```python
from build123d import *

# Parameters (mm, degrees)
SKETCH1_W                                            = 106
SKETCH1_H                                            = 187
BOSS_EXTRUDE1_DEPTH                                  = 9
SKETCH2_R                                            = 30
CUT_EXTRUDE1_DEPTH                                   = 109.973620661
SKETCH3_R                                            = 32.5
CUT_EXTRUDE2_DEPTH                                   = 7
CUT_EXTRUDE3_START                                   = -7
SKETCH4_R                                            = 32.5
CUT_EXTRUDE3_DEPTH                                   = 7
SKETCH5_W                                            = 62
SKETCH5_H                                            = 68
CUT_EXTRUDE4_DEPTH                                   = 109.973620661
FILLET1_R                                            = 2
SKETCH6_W                                            = 9
SKETCH6_H                                            = 87
CUT_EXTRUDE5_DEPTH                                   = 142.630681704
M4_TAPPED_HOLE1_D                                    = 3.3
M4_TAPPED_HOLE2_D                                    = 3.3
M3_TAPPED_HOLE1_D                                    = 2.5
M3_TAPPED_HOLE1_DEPTH                                = 7.5
M3_TAPPED_HOLE1_TIP                                  = 0.751075774
CHAMFER1_SIZE                                        = 5
HOLE_SIZE_PER_SOCKET_HEAD_CAP_SCREW_TYPE_D           = 4.5
HOLE_SIZE_PER_SOCKET_HEAD_CAP_SCREW_TYPE_CBORE_D     = 8
HOLE_SIZE_PER_SOCKET_HEAD_CAP_SCREW_TYPE_CBORE_DEPTH = 5
HOLE_SIZE_PER_SOCKET_HEAD_CAP_SCREW_2_D              = 5.5
HOLE_SIZE_PER_SOCKET_HEAD_CAP_SCREW_2_CBORE_D        = 10
HOLE_SIZE_PER_SOCKET_HEAD_CAP_SCREW_2_CBORE_DEPTH    = 9
M5_TAPPED_HOLE1_D                                    = 4.2
M5_TAPPED_HOLE1_DEPTH                                = 12.4
M5_TAPPED_HOLE1_TIP                                  = 1.2618073
M4_TAPPED_HOLE3_D                                    = 3.3
M4_TAPPED_HOLE3_DEPTH                                = 12.1
M4_TAPPED_HOLE3_TIP                                  = 0.991420021


with BuildPart() as part:
    # Sketch1 → Boss-Extrude1 (new, symmetric)
    with BuildSketch(Plane.XY):
        Rectangle(SKETCH1_W, SKETCH1_H)
    extrude(amount=BOSS_EXTRUDE1_DEPTH, both=True)

    # Sketch2 → Cut-Extrude1 (cut, through all)
    with BuildSketch(Plane(origin=(0, 0, -9), x_dir=(-1, 0, 0), z_dir=(0, 0, -1))):
        with Locations((0, 40.5)):
            Circle(SKETCH2_R)
    extrude(amount=-CUT_EXTRUDE1_DEPTH, mode=Mode.SUBTRACT)

    # Sketch3 → Cut-Extrude2 (cut)
    with BuildSketch(Plane.XY.offset(9)):
        with Locations((0, 40.5)):
            Circle(SKETCH3_R)
    extrude(amount=-CUT_EXTRUDE2_DEPTH, mode=Mode.SUBTRACT)

    # Sketch4 → Cut-Extrude3 (cut)
    with BuildSketch(Plane(origin=(0, 0, -9), x_dir=(-1, 0, 0), z_dir=(0, 0, -1)).offset(CUT_EXTRUDE3_START)):
        with Locations(Location((0, 40.5, 0), (0, 0, 180))):
            Circle(SKETCH4_R)
    extrude(amount=CUT_EXTRUDE3_DEPTH, mode=Mode.SUBTRACT)

    # Sketch5 → Cut-Extrude4 (cut, through all)
    with BuildSketch(Plane.XY.offset(9)):
        with Locations((0, -40.5)):
            Rectangle(SKETCH5_W, SKETCH5_H)
    extrude(amount=-CUT_EXTRUDE4_DEPTH, mode=Mode.SUBTRACT)

    # Fillet1
    fillet1_edges = [part.edges().sort_by_distance(p)[0] for p in [
        (-31, -74.5, 0),
        (-31, -6.5, 0),
        (31, -6.5, 0),
        (31, -74.5, 0),
    ]]
    fillet(fillet1_edges, radius=FILLET1_R)

    # Sketch6 → Cut-Extrude5 (cut, through all)
    with BuildSketch(Plane(origin=(53, 0, 0), x_dir=(0, 0, -1), z_dir=(1, 0, 0))):
        with Locations((-4.5, -50)):
            Rectangle(SKETCH6_W, SKETCH6_H)
    extrude(amount=-CUT_EXTRUDE5_DEPTH, mode=Mode.SUBTRACT)

    # M4 Tapped Hole1 (through all)
    with Locations(Plane.XY):
        with Locations((36, -24), (36, -59), (-36, -59), (-36, -24)):
            Hole(M4_TAPPED_HOLE1_D / 2)

    # M4 Tapped Hole2 (through all)
    with Locations(Plane.XY):
        with Locations((-8, -83.5), (8, -83.5)):
            Hole(M4_TAPPED_HOLE2_D / 2)

    # M3 Tapped Hole1
    with Locations(Plane.XY.offset(9)):
        with Locations((-38, 45.5), (-38, 37.5), (-38, -0.5)):
            Hole(M3_TAPPED_HOLE1_D / 2, depth=M3_TAPPED_HOLE1_DEPTH)
            with Locations((0, 0, -(M3_TAPPED_HOLE1_DEPTH + M3_TAPPED_HOLE1_TIP / 2))):  # 118° drill point
                Cone(0, M3_TAPPED_HOLE1_D / 2, M3_TAPPED_HOLE1_TIP, mode=Mode.SUBTRACT)

    # Chamfer1
    chamfer1_edges = [part.edges().sort_by_distance(p)[0] for p in [
        (-53, 93.5, 0),
        (53, 93.5, 0),
    ]]
    chamfer(chamfer1_edges, length=CHAMFER1_SIZE)

    # Hole size per socket head cap screw type (through all)
    with Locations(Plane(origin=(0, 0, -9), x_dir=(-1, 0, 0), z_dir=(0, 0, -1))):
        with Locations((-38, 33.5)):
            CounterBoreHole(HOLE_SIZE_PER_SOCKET_HEAD_CAP_SCREW_TYPE_D / 2, HOLE_SIZE_PER_SOCKET_HEAD_CAP_SCREW_TYPE_CBORE_D / 2, HOLE_SIZE_PER_SOCKET_HEAD_CAP_SCREW_TYPE_CBORE_DEPTH)

    # Hole size per socket head cap screw  2 (through all)
    with Locations(Plane.XY.offset(9)):
        with Locations((-47, 9.05741234), (-47, -30.94258766), (-47, -70.94258766), (47, -70.94258766), (47, -30.94258766), (47, 9.05741234)):
            CounterBoreHole(HOLE_SIZE_PER_SOCKET_HEAD_CAP_SCREW_2_D / 2, HOLE_SIZE_PER_SOCKET_HEAD_CAP_SCREW_2_CBORE_D / 2, HOLE_SIZE_PER_SOCKET_HEAD_CAP_SCREW_2_CBORE_DEPTH)

    # M5 Tapped Hole1
    with Locations(Plane.XY.offset(9)):
        with Locations((0, -0.5)):
            Hole(M5_TAPPED_HOLE1_D / 2, depth=M5_TAPPED_HOLE1_DEPTH)
            with Locations((0, 0, -(M5_TAPPED_HOLE1_DEPTH + M5_TAPPED_HOLE1_TIP / 2))):  # 118° drill point
                Cone(0, M5_TAPPED_HOLE1_D / 2, M5_TAPPED_HOLE1_TIP, mode=Mode.SUBTRACT)

    # M4 Tapped Hole3
    with Locations(Plane(origin=(0, 93.5, 0), x_dir=(1, 0, 0), z_dir=(0, 1, 0))):
        with Locations((-35, 0), (35, 0)):
            Hole(M4_TAPPED_HOLE3_D / 2, depth=M4_TAPPED_HOLE3_DEPTH)
            with Locations((0, 0, -(M4_TAPPED_HOLE3_DEPTH + M4_TAPPED_HOLE3_TIP / 2))):  # 118° drill point
                Cone(0, M4_TAPPED_HOLE3_D / 2, M4_TAPPED_HOLE3_TIP, mode=Mode.SUBTRACT)


solid = part.part
```
Can you work these out from the model? Positions are in its coordinate system, mm. A direction names the side the tool comes from. Give positions to 0.01 mm unless a question says otherwise; leave off trailing zeros. Loops run counter-clockwise (first coordinate to the right, second up) from the corner with the lowest first, then second, coordinate; pieces in that order, holes last. Notation, with made-up numbers: M -20.75,45.5 L -4.75,45.5 A21 cw -4.75,63.5 Z; hole C -38.5,81 d6. An arc over 180 degrees is marked long. One line per question, with ' | ' between items. Start each with the question number.
Q1. If we section it at D-D (x = 12.5): Please give me the cut outline in (y, z).
Q2. For faces 1 (the flat face through (1, -80, 0)), 2 (the flat face through (9.5, 11.8, 2)), 3 (the cylindrical face through (38.521, 37.466, -6.535)), 4 (the flat face through (31, -41, -4)), which set-ups out of +Z, -Z, +X, -X, +Y, -Y let a thin tool reach every point of the face, with its end or its side?
Q3. If we section it at C-C (y = 40.5): Please give me the cut outline in (x, z), plus the area to 3 significant figures.
Q4. If we section it at B-B (x = -26): Please give me the cut outline in (y, z).
Q5. If I drill on line 1 (Y direction, x = -38, z = 5.25); line 2 (Y direction, x = -36, z = -1.75); line 3 (Y direction, x = 0, z = 1.1), over which ranges is the centre line in solid material (lowest first)? Write a range as from..to.
Q6. For pin 1 Ø9 at (x, y) = (-47, -30.94) entering from +Z; pin 2 Ø3 at (x, z) = (-35, 0) entering from +Y; pin 3 Ø2 at (x, y) = (-38, 45.5) entering from +Z; pin 4 Ø2 at (x, y) = (-19, 21) entering from +Z, each with a flat end and sliding along its axis, tell me the tip position at first contact or that it passes through.
Q7. If we section it at A-A (y = -20): Please give me the cut outline in (x, z).
Q8. If we mould it in two halves opening along Y, with no side actions, what happens to faces 5 (the flat face through (-1, -93.5, -4)), 6 (the cylindrical face through (-7.6, -85.1, -4.6)), 7 (the flat face through (-1, 1, -9)), 8 (the flat face through (-1, 93.5, 0))? For each: +Y half, -Y half, draft (parallel to the pull), parting line (faces both ways), or undercut.
Computed:
1) outline: M -93.5,-9 L -74.5,-9 L -74.5,0 L -93.5,0 Z; M -6.5,-9 L 10.5,-9 L 10.5,-2 L 13.23,-2 L 13.23,2 L 10.5,2 L 10.5,9 L -6.5,9 Z; M 67.77,-2 L 70.5,-2 L 70.5,-9 L 93.5,-9 L 93.5,9 L 70.5,9 L 70.5,2 L 67.77,2 Z
2) face 1: +Z, +X, -X, -Y | face 2: +Z | face 3: -Z | face 4: +Z, -Z
3) outline: M -53,-9 L -32.5,-9 L -32.5,-2 L -30,-2 L -30,2 L -32.5,2 L -32.5,9 L -53,9 Z; M 30,-2 L 32.5,-2 L 32.5,-9 L 53,-9 L 53,9 L 32.5,9 L 32.5,2 L 30,2 Z | area: 758 mm²
4) outline: M -93.5,-9 L -74.5,-9 L -74.5,0 L -93.5,0 Z; M -6.5,-9 L 21,-9 L 21,-2 L 25.53,-2 L 25.53,2 L 21,2 L 21,9 L -6.5,9 Z; M 55.47,-2 L 60,-2 L 60,-9 L 93.5,-9 L 93.5,9 L 60,9 L 60,2 L 55.47,2 Z
5) line 1: y = -6.5..-1.75, 0.75..36.25, 38.75..44.25, 46.75..93.5 | line 2: y = -93.5..-60.65, -57.35..-25.65, -22.35..93.5 | line 3: y = -6.5..-2.6, 1.6..10.5, 70.5..93.5
6) pin 1: stops at z = 0 | pin 2: stops at y = 81.31 | pin 3: stops at z = 1.35 | pin 4: passes through
7) outline: M -53,-9 L -31,-9 L -31,0 L -53,0 Z; M 31,-9 L 53,-9 L 53,0 L 31,0 Z
8) face 5: -Y half | face 6: undercut | face 7: draft | face 8: +Y half
